Could you check a few things on this model? Use its own coordinates, in mm. Give positions to 0.01 mm unless a question says otherwise; leave off trailing zeros. Loops run counter-clockwise (first coordinate to the right, second up) from the corner with the lowest first, then second, coordinate; pieces in that order, holes last. Notation, with made-up numbers: M 3,-4 L 20,-4 A29 ccw 20,22 Z; hole C -36,26 d8. An arc over 180 degrees is marked long. Answer in a Markdown table with one row per item. Add a question column.
1. Thinking about a two-plate mould opening in Z: for faces 1 (the cylindrical face through (17, 0, 0)), 2 (the cylindrical face through (-13.905, 0.035, -0.867)), 3 (the flat face through (0, 2.5, 0)), which applies, released by +Z, released by -Z, zero draft, split by the parting line, or undercut?
2. If we section it at C-C on y = 1.45: List the corners of the cut face in (x, z) for me.
3. If we section it at D-D on z = 0: List the corners of the cut face in (x, y) for me.
4. I need wall thicknesses on line 1 along X through (y, z) = (-1.35, 0); line 2 along X through (y, z) = (1.3, -1.75); line 3 along X through (y, z) = (1.55, -5). Which ranges of each line are inside material? Lowest first, please. Write a range as from..to.
5. I'm going to push flat-ended pins straight in: pin 1 Ø1 at (y, z) = (-1, 3.5) entering from +X; pin 2 Ø1.5 at (y, z) = (1, 5) entering from -X. Where does each tip first touch, or does it pass through?
6. If we section it at B-B on x = 7: List the corners of the cut face in (y, z) for me, then the cut area to 3 significant figures.
7. If we section it at A-A on z = -2.5: List the corners of the cut face in (x, y) for me.
```python
from build123d import *

# Parameters (mm, degrees)
LINK_PLATE_DEPTH         = 2.5
HOLE_SKETCH_R            = 4
THROUGH_HOLES_2X_8_DEPTH = 2.5


with BuildPart() as part:
    # Link Profile Sketch → Link Plate (new, symmetric)
    with BuildSketch(Plane(origin=(0, 0, 0), x_dir=(1, 0, 0), z_dir=(0, 1, 0))):
        with BuildLine():
            Line((-10, 7), (10, 7))
            ThreePointArc((10, 7), (17, 0), (10, -7))
            Line((10, -7), (-10, -7))
            ThreePointArc((-10, -7), (-17, 0), (-10, 7))
        make_face()
    extrude(amount=LINK_PLATE_DEPTH, both=True)

    # Hole Sketch → Through Holes 2xØ8 (cut, symmetric)
    with BuildSketch(Plane(origin=(0, 0, 0), x_dir=(1, 0, 0), z_dir=(0, 1, 0))):
        with Locations(Location((10, 0, 0), (0, 0, 270))):
            Circle(HOLE_SKETCH_R)
        with Locations(Location((-10, 0, 0), (0, 0, 270))):
            Circle(HOLE_SKETCH_R)
    extrude(amount=THROUGH_HOLES_2X_8_DEPTH, both=True, mode=Mode.SUBTRACT)


solid = part.part
```
Results:
| question | item | result |
|---|---|---|
| 1 | face 1 | split by the parting line |
| 1 | face 2 | undercut |
| 1 | face 3 | zero draft |
| 2 | outline | M -10,-7 L 10,-7 A7 ccw 10,7 L -10,7 A7 ccw Z; hole C -10,0 d8; hole C 10,0 d8 |
| 3 | outline | M -17,-2.5 L -14,-2.5 L -14,2.5 L -17,2.5 Z; M -6,-2.5 L 6,-2.5 L 6,2.5 L -6,2.5 Z; M 14,-2.5 L 17,-2.5 L 17,2.5 L 14,2.5 Z |
| 4 | line 1 | -17..-14, -6..6, 14..17 |
| 4 | line 2 | -16.78..-13.6, -6.4..6.4, 13.6..16.78 |
| 4 | line 3 | -14.9..14.9 |
| 5 | pin 1 | x = 16.32 |
| 5 | pin 2 | x = -15.56 |
| 6 | outline | M -2.5,-7 L 2.5,-7 L 2.5,-2.65 L -2.5,-2.65 Z; M -2.5,2.65 L 2.5,2.65 L 2.5,7 L -2.5,7 Z |
| 6 | area | 43.5 mm2 |
| 7 | outline | M -16.54,-2.5 L -13.12,-2.5 L -13.12,2.5 L -16.54,2.5 Z; M -6.88,-2.5 L 6.88,-2.5 L 6.88,2.5 L -6.88,2.5 Z; M 13.12,-2.5 L 16.54,-2.5 L 16.54,2.5 L 13.12,2.5 Z |
